from build123d import *

# Parameters (mm, degrees)
SKETCH1_W           = 770
SKETCH1_H           = 80
BOSS_EXTRUDE1_DEPTH = 80
SKETCH3_W           = 5
SKETCH3_H           = 80
BOSS_EXTRUDE2_DEPTH = 70
SKETCH4_W           = 5
SKETCH4_H           = 80
BOSS_EXTRUDE3_DEPTH = 70
FILLET2_R           = 10
CUT_EXTRUDE1_DEPTH  = 690.814789958


with BuildPart() as part:
    # Sketch1 → Boss-Extrude1 (new body)
    with BuildSketch(Plane(origin=(0, 30, 0), x_dir=(1, 0, 0), z_dir=(0, 1, 0))):
        with Locations((228.333333333, 0)):
            Rectangle(SKETCH1_W, SKETCH1_H)
    extrude(amount=-BOSS_EXTRUDE1_DEPTH)

    # Sketch3 → Boss-Extrude2 (add)
    with BuildSketch(Plane.ZY.offset(156.666666667)):
        with Locations((37.5, -10)):
            Rectangle(SKETCH3_W, SKETCH3_H)
    extrude(amount=BOSS_EXTRUDE2_DEPTH)

    # Sketch4 → Boss-Extrude3 (add)
    with BuildSketch(Plane(origin=(613.333333333, 0, 0), x_dir=(0, 0, -1), z_dir=(1, 0, 0))):
        with Locations((-37.5, -10)):
            Rectangle(SKETCH4_W, SKETCH4_H)
    extrude(amount=BOSS_EXTRUDE3_DEPTH)

    # Fillet2
    fillet2_edges = [part.edges().sort_by_distance(p)[0] for p in [
        (228.333333333, 30, 40),
        (228.333333333, -50, 40),
        (228.333333333, -50, -40),
        (228.333333333, 30, -40),
    ]]
    fillet(fillet2_edges, radius=FILLET2_R)

    # Sketch6 → Cut-Extrude1 (cut, through all)
    with BuildSketch(Plane.XY.offset(40)):
        with BuildLine():
            Line((-206.666666667, -24), (-186.666666667, -24))
            ThreePointArc((-186.666666667, -24), (-180.666666667, -30), (-186.666666667, -36))
            Line((-186.666666667, -36), (-206.666666667, -36))
            ThreePointArc((-206.666666667, -36), (-212.666666667, -30), (-206.666666667, -24))
        make_face()
        with BuildLine():
            Line((-206.666666667, 16), (-186.666666667, 16))
            ThreePointArc((-186.666666667, 16), (-180.666666667, 10), (-186.666666667, 4))
            Line((-186.666666667, 4), (-206.666666667, 4))
            ThreePointArc((-206.666666667, 4), (-212.666666667, 10), (-206.666666667, 16))
        make_face()
        with BuildLine():
            Line((663.333333333, 16), (643.333333333, 16))
            ThreePointArc((643.333333333, 16), (637.333333333, 10), (643.333333333, 4))
            Line((643.333333333, 4), (663.333333333, 4))
            ThreePointArc((663.333333333, 4), (669.333333333, 10), (663.333333333, 16))
        make_face()
        with BuildLine():
            Line((663.333333333, -24), (643.333333333, -24))
            ThreePointArc((643.333333333, -24), (637.333333333, -30), (643.333333333, -36))
            Line((643.333333333, -36), (663.333333333, -36))
            ThreePointArc((663.333333333, -36), (669.333333333, -30), (663.333333333, -24))
        make_face()
    extrude(amount=-CUT_EXTRUDE1_DEPTH, mode=Mode.SUBTRACT)


solid = part.part
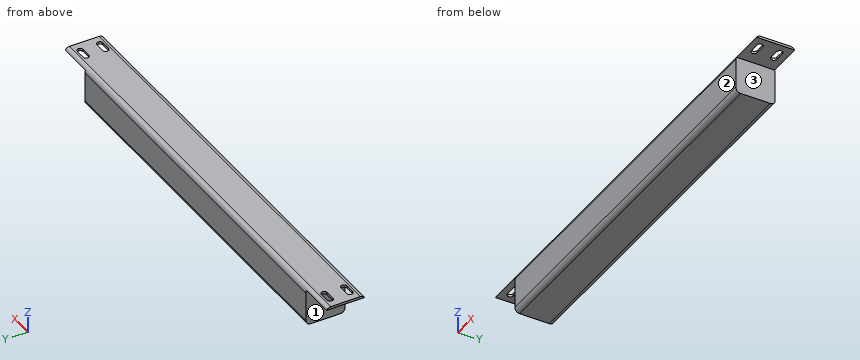
Model file for the job. Use its own axes, mm. Face numbers are marked on the shaded views. A direction names the side the tool comes from. Give positions to 0.01 mm unless a question says otherwise; leave off trailing zeros. Loops run counter-clockwise (first coordinate to the right, second up) from the corner with the lowest first, then second, coordinate; pieces in that order, holes last. Notation, with made-up numbers: (48, -24.75) -> (104, -24.75) arc R19 ccw to (104, -6.75) -> close; hole circle Ø7 at (-13.5, 61). An arc over 180 degrees is marked (long way). Use a Markdown table: item, result. Add a question column.
(1) Drop flat-ended pins along their axis: pin 1 Ø5.5 at (x, z) = (-197, 37) entering from -Y; pin 2 Ø4 at (x, z) = (-199, 37.5) entering from -Y; pin 3 Ø8 at (y, z) = (-23.5, -1.5) entering from +X. Give the stop position or say it passes through.
(2) Tool access for the marked faces 1, 2 and 3: list every direction of +Z, -Z, +X, -X, +Y, -Y with a clear straight run to the whole face (end or side of a thin tool).
(3) Slice it at A-A on z = 20. List the corners of the cut face in (x, y), and give its area (3 significant figures).
(4) Wall check: line 1 along X through (y, z) = (20, 17); line 2 along Z through (x, y) = (621, 15); line 3 along Y through (x, z) = (371.5, -34). Give the ranges that are in metal, low to high.
Filled sheet:
| question | item | result |
|---|---|---|
| 1 | pin 1 | y = -48.66 |
| 1 | pin 2 | y = -48.35 |
| 1 | pin 3 | x = 613.33 |
| 2 | face 1 | -Z, -X, +Y, -Y |
| 2 | face 2 | +Z, -Z, +X, -X, -Y |
| 2 | face 3 | -Z, +X, +Y, -Y |
| 3 | outline | (-156.67, -50) -> (613.33, -50) -> (613.33, 30) -> (-156.67, 30) -> close |
| 3 | area | 61,600 mm2 |
| 4 | line 1 | -156.67 to 613.33 |
| 4 | line 2 | 35 to 40 |
| 4 | line 3 | -49.17 to 29.17 |
